Build history of the part. All positions in model axes, mm. Round coordinates to 2 decimals unless told otherwise and drop trailing zeros. Order: outer loops, then holes, each group sorted by start corner. A loop starts at its lowest first (then second) coordinate and runs counter-clockwise, first axis right, second up. Notation, with made-up numbers: M 74,-1 L 113,-1 A13 ccw 113,19 Z; hole C -16,-14 d4. An arc over 180 degrees is marked long. One line per item, written item: value. Start each with the question number.
Item 1: Band-saw the part on C-C, the plane x = 1454. Write the cut outline in (y, z).
Item 2: Band-saw the part on B-B, the plane y = 467.5. Write the cut outline in (x, z), then the cut area to 3 significant figures.
Item 3: Probe L1, parallel to X at y = 1142, z = 1.25; L2, parallel to X at y = 1096, z = -0.5; L3, parallel to Y at x = 1297.5, z = 0. List the from-to ranges inside material, lowest first.
Item 4: Band-saw the part on A-A, the plane z = 0. Write the cut outline in (x, y).
Item 5: Pin check, flat tips, straight feed: pin 1 (3 mm diameter, centred on y = 1030, z = 0.5, fed in from -X); pin 2 (1 mm diameter, centred on x = 1406.5, z = 2, fed in from -Y); pin 3 (1.5 mm diameter, centred on y = 709.5, z = -2, fed in from -X). Stop position of each tip, or through.
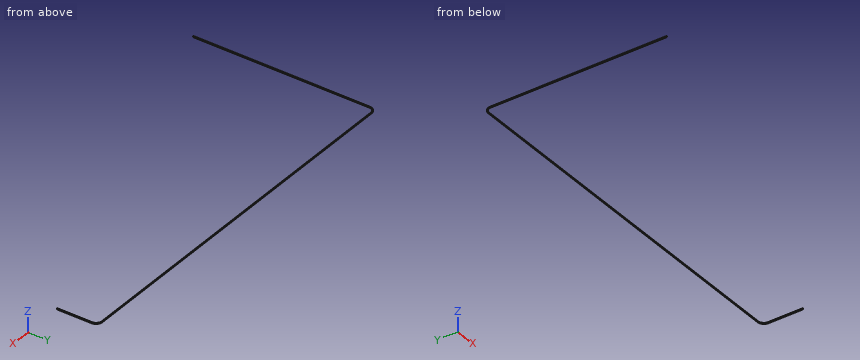
```python
from build123d import *

# Parameters (mm, degrees)
SKETCH2_R = 3.25


with BuildPart() as part:
    # Sweep1: sweep along a path in Sketch1
    with BuildLine(Plane.XY) as sweep1_path:
        Line((0, 0), (0, 1213))
        ThreePointArc((0, 1213), (12.30151519, 1242.69848481), (42, 1255))
        Line((42, 1255), (2620, 1255))
        ThreePointArc((2620, 1255), (2649.69848481, 1242.69848481), (2662, 1213))
        Line((2662, 1213), (2662, 975))
    # Sketch2 → Sweep1 (sweep)
    with BuildSketch(Plane(origin=(0, 0, 0), x_dir=(1, 0, 0), z_dir=(0, 1, 0))):
        Circle(SKETCH2_R)
    sweep(path=sweep1_path.line)


solid = part.part
```
Output:
1. outline: C 1255,0 d6.5
2. outline: C 0,0 d6.5
2. area: 33.2 mm²
3. L1: x = -3 to 3, 2659 to 2665
3. L2: x = -3.21 to 3.21, 2658.79 to 2665.21
3. L3: y = 1251.75 to 1258.25
4. outline: M -3.25,0 L 3.25,0 L 3.25,1213 A38.75 cw 42,1251.75 L 2620,1251.75 A38.75 cw 2658.75,1213 L 2658.75,975 L 2665.25,975 L 2665.25,1213 A45.25 ccw 2620,1258.25 L 42,1258.25 A45.25 ccw -3.25,1213 Z
5. pin 1: stops at x = -3.25
5. pin 2: stops at y = 1252.12
5. pin 3: stops at x = -3
